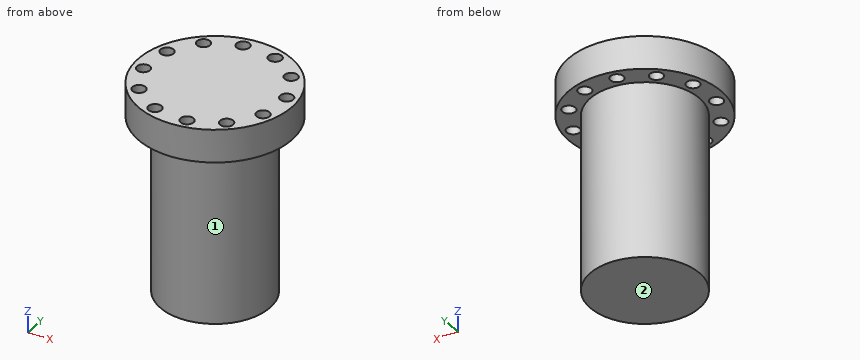
```python
from build123d import *

# Parameters (mm, degrees)
SKETCH1_R               = 17.5
BOSS_EXTRUDE1_DEPTH     = 7.5
SKETCH2_R               = 12.5
BOSS_EXTRUDE2_DEPTH     = 40
CUT_EXTRUDE1_DEPTH      = 109.253175473
CUT_EXTRUDE1_DEPTH_BACK = 109.253175473
SKETCH3_R               = 1.5


with BuildPart() as part:
    # Sketch1 → Boss-Extrude1 (new body)
    with BuildSketch(Plane.XY):
        with Locations((-70, 25)):
            Circle(SKETCH1_R)
    extrude(amount=BOSS_EXTRUDE1_DEPTH)

    # Sketch2 → Boss-Extrude2 (add)
    with BuildSketch(Plane(origin=(0, 0, 0), x_dir=(-1, 0, 0), z_dir=(0, 0, -1))):
        with Locations((70, 25)):
            Circle(SKETCH2_R)
    extrude(amount=BOSS_EXTRUDE2_DEPTH)

    # Sketch3 → Cut-Extrude1 (cut, two sides: drawn at the far end of the back side and taken through both)
    with BuildSketch(Plane.XY.offset(7.5).offset(-CUT_EXTRUDE1_DEPTH_BACK)):
        with Locations((-81.608310906, 15.50015169)):
            Circle(SKETCH3_R)
        with Locations((-84.803016294, 22.577045484)):
            Circle(SKETCH3_R)
        with Locations((-84.031265422, 30.303167984)):
            Circle(SKETCH3_R)
        with Locations((-79.49984831, 36.608310906)):
            Circle(SKETCH3_R)
        with Locations((-72.422954516, 39.803016294)):
            Circle(SKETCH3_R)
        with Locations((-64.696832016, 39.031265422)):
            Circle(SKETCH3_R)
        with Locations((-58.391689094, 34.49984831)):
            Circle(SKETCH3_R)
        with Locations((-55.196983706, 27.422954516)):
            Circle(SKETCH3_R)
        with Locations((-55.968734578, 19.696832016)):
            Circle(SKETCH3_R)
        with Locations((-60.50015169, 13.391689094)):
            Circle(SKETCH3_R)
        with Locations((-67.577045484, 10.196983706)):
            Circle(SKETCH3_R)
        with Locations((-75.303167984, 10.968734578)):
            Circle(SKETCH3_R)
    extrude(amount=CUT_EXTRUDE1_DEPTH + CUT_EXTRUDE1_DEPTH_BACK, mode=Mode.SUBTRACT)


solid = part.part
```
Input: part model. Units: mm. Frame: model coordinates. Face numbers are marked on the shaded views. A direction names the side the tool comes from. Coordinates: 2 decimals unless noted, no trailing zeros. Loops run counter-clockwise (first coordinate to the right, second up) from the corner with the lowest first, then second, coordinate; pieces in that order, holes last.
Q1. Set-up query: the marked faces 1 and 2. Return all of +Z, -Z, +X, -X, +Y, -Y with unobstructed straight access to the full face (end or side cutting, diameter ignored); none if empty.
Results are:
face 1: -Z
face 2: -Z, +X, -X, +Y, -Y
Q2. Section C-C, the plane z = -20. Return the cut outline in (x, y).
Results are:
outline: circle Ø25 at (-70, 25)
Q3. Line query: line 1 along Z through (x, y) = (-56.5, 36); line 2 along X through (y, z) = (24.5, -31); line 3 along X through (y, z) = (31.5, -12). Output: solid intervals per line, ascending.
Results are:
line 1: z = 0 to 7.5
line 2: x = -82.49 to -57.51
line 3: x = -80.68 to -59.32
Q4. Section A-A, the plane x = -61. Return the cut outline in (y, z).
Results are:
outline: (9.99, 0) - (11.98, 0) - (11.98, 7.5) - (9.99, 7.5) - close; (14.81, 0) - (16.33, 0) - (16.33, -40) - (33.67, -40) - (33.67, 0) - (40.01, 0) - (40.01, 7.5) - (14.81, 7.5) - close
Q5. Contact query for flat-ended pins moving along their axis: pin 1 (2.5 mm diameter, centred on x = -58.39, y = 34.5, fed in from +Z); pin 2 (3.5 mm diameter, centred on x = -60.5, y = 13.39, fed in from -Z); pin 3 (12 mm diameter, centred on y = 16.5, z = -28, fed in from -X); pin 4 (6 mm diameter, centred on x = -62, z = -3.5, fed in from -Y). Output: stop coordinate, or through.
Results are:
pin 1: passes through
pin 2: stops at z = 0
pin 3: stops at x = -82.25
pin 4: stops at y = 13.54
Q6. Section B-B, the plane x = -70. Return the cut outline in (y, z).
Results are:
outline: (7.5, 0) - (12.5, 0) - (12.5, -40) - (37.5, -40) - (37.5, 0) - (42.5, 0) - (42.5, 7.5) - (7.5, 7.5) - close
